from build123d import *

# Parameters (mm, degrees)
SKETCH1_R           = 42.5
SKETCH1_R_2         = 30.25
BOSS_EXTRUDE1_DEPTH = 3
SKETCH2_R           = 2.4
CUT_EXTRUDE1_DEPTH  = 3


with BuildPart() as part:
    # Sketch1 → Boss-Extrude1 (new body)
    with BuildSketch(Plane.XY):
        Circle(SKETCH1_R)
        Circle(SKETCH1_R_2, mode=Mode.SUBTRACT)
    extrude(amount=BOSS_EXTRUDE1_DEPTH)

    # Sketch2 → Cut-Extrude1 (cut)
    with BuildSketch(Plane.XY.offset(3)):
        with Locations((0, 37)):
            Circle(SKETCH2_R)
        with Locations((32.04293994, 18.5)):
            Circle(SKETCH2_R)
        with Locations((32.04293994, -18.5)):
            Circle(SKETCH2_R)
        with Locations((0, -37)):
            Circle(SKETCH2_R)
        with Locations((-32.04293994, -18.5)):
            Circle(SKETCH2_R)
        with Locations((-32.04293994, 18.5)):
            Circle(SKETCH2_R)
    extrude(amount=-CUT_EXTRUDE1_DEPTH, mode=Mode.SUBTRACT)


solid = part.part
Input: part model. Units: mm. Frame: model coordinates. Give positions to 0.01 mm unless a question says otherwise; leave off trailing zeros. Loops run counter-clockwise (first coordinate to the right, second up) from the corner with the lowest first, then second, coordinate; pieces in that order, holes last. Notation, with made-up numbers: (-26.75, 53.25) - (-0.75, 53.25) arc R19 cw to (-0.75, 78.25) - close; hole circle Ø1 at (65.5, 29). An arc over 180 degrees is marked (long way). Use CSV: the item, a comma, the result in double quotes. Start each with the question number.
Item 1: Mould query, pull axis Y, two halves, no side actions, for faces 1 (the cylindrical face through (34.26, -19.42, 1.52)), 2 (the flat face through (-10, 29, 0)), 3 (the cylindrical face through (-33.727, -25.861, 1.479)). Classes: pulls with the +Y half, pulls with the -Y half, needs draft (parallel to the pull), parting line crosses it, or undercut.
Item 2: Contact query for flat-ended pins moving along their axis: P1, Ø1, axis at x = 15.5, z = 2.5, coming from the -Y side; P2, Ø4, axis at x = -32.04, y = -18.5, coming from the -Z side; P3, Ø1.5, axis at y = 7.5, z = 1, coming from the -X side; P4, Ø1, axis at y = -8, z = 2, coming from the +X side. Output: stop coordinate, or through.
Item 3: Section A-A on y = 0. Return loops of the section in (x, z), then the cut area to 3 significant figures.
Item 4: Section B-B on x = 0. Return loops of the section in (y, z).
Item 5: Section C-C on z = 0.95. Return loops of the section in (x, y), then the cut area to 3 significant figures.
Item 6: Line query: line 1 (Y direction, x = 0, z = 2.45); line 2 (X direction, y = 17, z = 1.2); line 3 (X direction, y = -0.5, z = 1.4). Output: solid intervals per line, ascending.
Item 7: Section D-D on y = -18.5. Return loops of the section in (x, z), then the cut area to 3 significant figures.
Ans:
1,face 1,"undercut"
1,face 2,"needs draft"
1,face 3,"parting line crosses it"
2,P1,"stops at y = -39.76"
2,P2,"passes through"
2,P3,"stops at x = -41.96"
2,P4,"stops at x = 41.83"
3,outline,"(-42.5, 0) - (-30.25, 0) - (-30.25, 3) - (-42.5, 3) - close; (30.25, 0) - (42.5, 0) - (42.5, 3) - (30.25, 3) - close"
3,area,"73.5 mm2"
4,outline,"(-42.5, 0) - (-39.4, 0) - (-39.4, 3) - (-42.5, 3) - close; (-34.6, 0) - (-30.25, 0) - (-30.25, 3) - (-34.6, 3) - close; (30.25, 0) - (34.6, 0) - (34.6, 3) - (30.25, 3) - close; (39.4, 0) - (42.5, 0) - (42.5, 3) - (39.4, 3) - close"
5,outline,"circle Ø85 at (0, 0); hole circle Ø4.8 at (-32.04, -18.5); hole circle Ø4.8 at (-32.04, 18.5); hole circle Ø60.5 at (0, 0); hole circle Ø4.8 at (0, -37); hole circle Ø4.8 at (0, 37); hole circle Ø4.8 at (32.04, -18.5); hole circle Ø4.8 at (32.04, 18.5)"
5,area,"2,690 mm2"
6,line 1,"y = -42.5 to -39.4, -34.6 to -30.25, 30.25 to 34.6, 39.4 to 42.5"
6,line 2,"x = -38.95 to -33.92, -30.17 to -25.02, 25.02 to 30.17, 33.92 to 38.95"
6,line 3,"x = -42.5 to -30.25, 30.25 to 42.5"
7,outline,"(-38.26, 0) - (-34.44, 0) - (-34.44, 3) - (-38.26, 3) - close; (-29.64, 0) - (-23.93, 0) - (-23.93, 3) - (-29.64, 3) - close; (23.93, 0) - (29.64, 0) - (29.64, 3) - (23.93, 3) - close; (34.44, 0) - (38.26, 0) - (38.26, 3) - (34.44, 3) - close"
7,area,"57.2 mm2"
